from build123d import *


with BuildPart() as part:
    # 草图1 → 旋转1 (revolve)
    with BuildSketch(Plane.XY, mode=Mode.PRIVATE) as revolve_1_sk:
        Polygon((0, 2.646643634), (2, 2.646643634), (2, 1.646643634), (1.9, 1.646643634), (1.9, 1.046643634), (2, 1.046643634), (2, -10.953356366), (1.9, -10.953356366), (1.9, -11.553356366), (2, -11.553356366), (2, -12.553356366), (0, -12.553356366), align=None)
    revolve(revolve_1_sk.sketch.rotate(Axis((0, 2.646643634, 0), (0, -1, 0)), 180), axis=Axis((0, 2.646643634, 0), (0, -1, 0)))


solid = part.part
Verification items for the finished model (mm, model axes). Give positions to 0.01 mm unless a question says otherwise; leave off trailing zeros. Order: outer loops, then holes, each group sorted by start corner. A loop starts at its lowest first (then second) coordinate and runs counter-clockwise, first axis right, second up. Notation, with made-up numbers: M 48.5,52 L 75.5,52 A6 cw 75.5,56 Z; hole C -31.5,15 d5. An arc over 180 degrees is marked long. Answer as a JSON object with one key per item and string values. Group by question number.
1) Mould release check, pull along Y, two halves, no side actions. Record for faces 1 (the face through (-1.812, -11.258, -0.571)), 2 (the face through (0, 2.647, 0)), 3 (the face through (-1.812, 1.342, -0.571)), 4 (the face through (0, -12, 2)): released by +Y, released by -Y, zero draft, split by the parting line, or undercut.
2) Scan lines: line 1 along X through (y, z) = (-7, 0.8); line 2 along Z through (x, y) = (-1.4, -4.5); line 3 along X through (y, z) = (-3.5, -1.7). Record each from-to range of solid material in increasing order. Write a range as [from, to].
3) Cross-section at B-B (z = -1.35). Enter the section's corners in (x, y), then the cut area to 3 significant figures.
4) Cross-section at A-A (x = 1.65). Enter the section's corners in (y, z), then the cut area to 3 significant figures.
5) Cross-section at C-C (y = -6). Enter the section's corners in (x, z).
Result sheet:
{
 "1": {"face 1": "undercut", "face 2": "released by +Y", "face 3": "undercut", "face 4": "zero draft"},
 "2": {"line 1": "x = [-1.83, 1.83]", "line 2": "z = [-1.43, 1.43]", "line 3": "x = [-1.05, 1.05]"},
 "3": {"outline": "M -1.48,-12.55 L 1.48,-12.55 L 1.48,-11.55 L 1.34,-11.55 L 1.34,-10.95 L 1.48,-10.95 L 1.48,1.05 L 1.34,1.05 L 1.34,1.65 L 1.48,1.65 L 1.48,2.65 L -1.48,2.65 L -1.48,1.65 L -1.34,1.65 L -1.34,1.05 L -1.48,1.05 L -1.48,-10.95 L -1.34,-10.95 L -1.34,-11.55 L -1.48,-11.55 Z", "area": "44.5 mm2"},
 "4": {"outline": "M -12.55,-1.13 L -11.55,-1.13 L -11.55,-0.94 L -10.95,-0.94 L -10.95,-1.13 L 1.05,-1.13 L 1.05,-0.94 L 1.65,-0.94 L 1.65,-1.13 L 2.65,-1.13 L 2.65,1.13 L 1.65,1.13 L 1.65,0.94 L 1.05,0.94 L 1.05,1.13 L -10.95,1.13 L -10.95,0.94 L -11.55,0.94 L -11.55,1.13 L -12.55,1.13 Z", "area": "33.9 mm2"},
 "5": {"outline": "C 0,0 d4"}
}
